Work out the finished part from the listing and answer in its coordinate system (mm). Face numbers are marked on the shaded views. A direction names the side the tool comes from. Round coordinates to 2 decimals unless told otherwise and drop trailing zeros. Loops run counter-clockwise (first coordinate to the right, second up) from the corner with the lowest first, then second, coordinate; pieces in that order, holes last. Notation, with made-up numbers: (73, 13) - (96, 13) arc R7 ccw to (96, 24) - close; hole circle Ø3 at (34.5, 72.5). An arc over 180 degrees is marked (long way). Answer as CSV lines item,"result". Start each with the question number.
Q1. The mould has two halves that part along X. Classify the marked faces 1, 2, 3 and 4: +X half, -X half, draft (parallel to the pull), parting line (faces both ways), or undercut.
Q2. Each of these flat-tipped pins is pushed along its axis until it touches: pin 1 Ø1 at (y, z) = (66.5, 14) entering from -X; pin 2 Ø9.5 at (y, z) = (5.5, -10) entering from +X; pin 3 Ø1 at (x, z) = (-7.5, -20.5) entering from +Y; pin 4 Ø2 at (x, y) = (-9.5, 31) entering from -Z. Where does it stop, or does it pass through?
Q3. Section D-D on z = 3 is taken. Write down the section's boundary in (x, y).
Q4. Section A-A on x = -16 is taken. Write down the section's boundary in (y, z), then the cut area to 3 significant figures.
Q5. Section C-C on x = 2 is taken. Write down the section's boundary in (y, z), then the cut area to 3 significant figures.
Q6. For the marked faces 5, 6 and 7, determine the directions among +Z, -Z, +X, -X, +Y, -Y from which every point of the face is accessible in a straight line to the end or side of a thin tool.
Q7. Straight lines are drawn through the part: L1, parallel to Z at x = -11, y = 20; L2, parallel to X at y = 25, z = 25; L3, parallel to Z at x = 0, y = 7. For each, find the intervals that lie inside material, in ascending order. Write a range as [from, to].
Q8. Section B-B on y = 32 is taken. Write down the section's boundary in (x, z), then the cut area to 3 significant figures.
```python
from build123d import *

# Parameters (mm, degrees)
UPRIGHT_LUG_SKETCH_R     = 8
UPRIGHT_LUG_DEPTH        = 12
CLEVIS_SIDE_LUG_SKETCH_R = 8
CLEVIS_SIDE_LUG_DEPTH    = 12
HORIZONTAL_LUG_SKETCH_R  = 8
HORIZONTAL_LUG_DEPTH     = 12


with BuildPart() as part:
    # Upright Lug Sketch → Upright Lug (new body)
    with BuildSketch(Plane.XY):
        with BuildLine():
            Line((-20, 0), (20, 0))
            Line((20, 0), (20, 60))
            ThreePointArc((20, 60), (0, 80), (-20, 60))
            Line((-20, 60), (-20, 0))
        make_face()
        with Locations((0, 60)):
            Circle(UPRIGHT_LUG_SKETCH_R, mode=Mode.SUBTRACT)
    extrude(amount=UPRIGHT_LUG_DEPTH)

    # Clevis Side Lug Sketch → Clevis Side Lug (add)
    with BuildSketch(Plane(origin=(20, 0, 0), x_dir=(0, 0, -1), z_dir=(1, 0, 0))):
        with BuildLine():
            Line((0, 0), (-40, 0))
            ThreePointArc((-40, 0), (-60, 20), (-40, 40))
            Line((-40, 40), (0, 40))
            Line((0, 40), (0, 0))
        make_face()
        with Locations(Location((-40, 20, 0), (0, 0, 90))):
            Circle(CLEVIS_SIDE_LUG_SKETCH_R, mode=Mode.SUBTRACT)
    clevis_side_lug = extrude(amount=-CLEVIS_SIDE_LUG_DEPTH)

    # Clevis Side Lug Mirror: Clevis Side Lug across plane
    add(clevis_side_lug.mirror(Plane(origin=(0, 0, 0), x_dir=(0, 0, 1), z_dir=(1, 0, 0))))

    # Horizontal Lug Sketch → Horizontal Lug (add)
    with BuildSketch(Plane.XZ):
        with BuildLine():
            Line((-20, 12), (19.961751116, 12))
            Line((19.961751116, 12), (19.961751116, -25.763677886))
            ThreePointArc((19.961751116, -25.763677886), (0.618456819, -46.990435492), (-20, -27))
            Line((-20, -27), (-20, 12))
        make_face()
        with Locations((0, -27)):
            Circle(HORIZONTAL_LUG_SKETCH_R, mode=Mode.SUBTRACT)
    extrude(amount=-HORIZONTAL_LUG_DEPTH)


solid = part.part
```
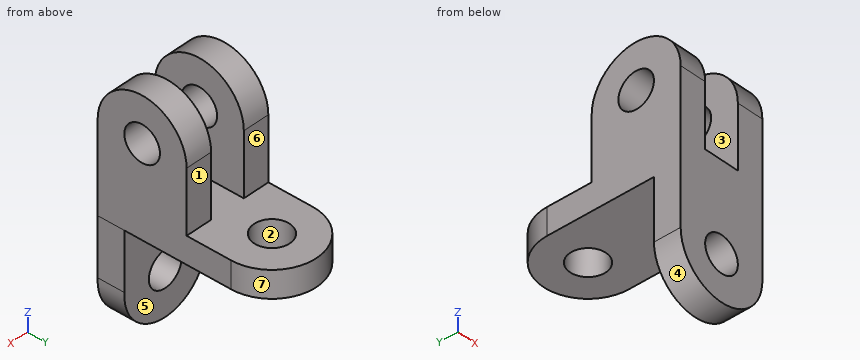
Findings:
1,face 1,"draft"
1,face 2,"undercut"
1,face 3,"undercut"
1,face 4,"parting line"
2,pin 1,"passes through"
2,pin 2,"stops at x = 19.96"
2,pin 3,"stops at y = 12"
2,pin 4,"stops at z = 0"
3,outline,"(-20, 0) - (20, 0) - (20, 60) arc R20 ccw to (-20, 60) - close; hole circle Ø16 at (0, 60)"
4,outline,"(0, -39) - (12, -39) - (12, 0) - (72, 0) - (72, 12) - (40, 12) - (40, 40) arc R20 ccw to (0, 40) - close; hole circle Ø16 at (20, 40)"
4,area,"2,880 mm^2"
5,outline,"(0, -46.9) - (12, -46.9) - (12, -34.75) - (0, -34.75) - close; (0, -19.25) - (12, -19.25) - (12, 0) - (52.25, 0) - (52.25, 12) - (0, 12) - close; (67.75, 0) - (79.9, 0) - (79.9, 12) - (67.75, 12) - close"
5,area,"1,150 mm^2"
6,face 5,"-Z, +X, -X, +Y"
6,face 6,"+Z, +X, -X, +Y"
6,face 7,"+Z, -Z, +Y"
7,L1,"z = [0, 32], [48, 60]"
7,L2,"x = [-20, -8], [8, 20]"
7,L3,"z = [-47, -35], [-19, 12]"
8,outline,"(-20, 0) - (20, 0) - (20, 56) - (8, 56) - (8, 12) - (-8, 12) - (-8, 56) - (-20, 56) - close"
8,area,"1,540 mm^2"
